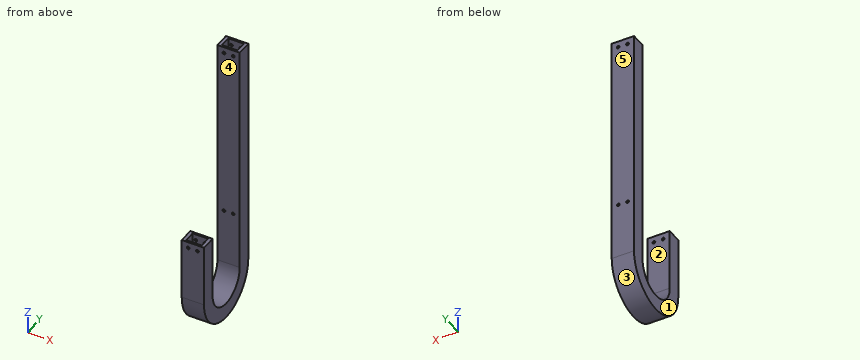
```python
from build123d import *

# Parameters (mm, degrees)
SKETCH_2_W          = 36
SKETCH_2_H          = 24
SKETCH_2_W_2        = 25
SKETCH_2_H_2        = 18
SKETCH_4_R          = 2.25
CUT_EXTRUDE_1_DEPTH = 304.110540892


with BuildPart() as part:
    # 扫描1: sweep along a path in 草图3
    with BuildLine(Plane(origin=(0, 0, 0), x_dir=(0, 0, -1), z_dir=(1, 0, 0))) as sweep_1_path:
        Line((0, 0), (100, 0))
        ThreePointArc((100, 0), (150, 50), (100, 100))
        Line((100, 100), (-276, 100))
    # 草图2 → 扫描1 (sweep)
    with BuildSketch(Plane.XY):
        Rectangle(SKETCH_2_W, SKETCH_2_H)
        Rectangle(SKETCH_2_W_2, SKETCH_2_H_2, mode=Mode.SUBTRACT)
    sweep(path=sweep_1_path.line)

    # 草图4 → 切除-拉伸1 (cut, through all)
    with BuildSketch(Plane.XZ.offset(12)):
        with Locations(Location((-7.5, -10, 0), (0, 0, 180))):
            Circle(SKETCH_4_R)
        with Locations(Location((7.5, -10, 0), (0, 0, 180))):
            Circle(SKETCH_4_R)
        with Locations(Location((-7.5, 266, 0), (0, 0, 270))):
            Circle(SKETCH_4_R)
        with Locations(Location((7.5, 266, 0), (0, 0, 270))):
            Circle(SKETCH_4_R)
    extrude(amount=-CUT_EXTRUDE_1_DEPTH, mode=Mode.SUBTRACT)


solid = part.part
```
Could you check a few things on this model? Use its own coordinates, in mm. Face numbers are marked on the shaded views. A direction names the side the tool comes from. Round coordinates to 2 decimals unless told otherwise and drop trailing zeros. Loops run counter-clockwise (first coordinate to the right, second up) from the corner with the lowest first, then second, coordinate; pieces in that order, holes last. Notation, with made-up numbers: M 20.25,23.5 L 45.25,23.5 A14 cw 45.25,36.5 Z; hole C -17,5 d5. An arc over 180 degrees is marked long. Answer as CSV lines item,"result".
1) Imagine slicing it at C-C on z = 244.5. List the corners of the cut face in (x, y) for me.
From the geometry:
outline,"M -18,88 L 18,88 L 18,112 L -18,112 Z; hole M -12.5,91 L 12.5,91 L 12.5,109 L -12.5,109 Z"
2) Which directions (+Z, -Z, +X, -X, +Y, -Y) give clear straight access to the entire face, cutting with the end or side of a thin tool? Please do the marked faces 1 and 2.
From the geometry:
face 1,"+Z, -Z, -X, +Y, -Y"
face 2,"+Z, +X, -X"
3) Imagine slicing it at D-D on y = -3. List the corners of the cut face in (x, z) for me, and give its area (3 significant figures).
From the geometry:
outline,"M -18,-132.17 L 18,-132.17 L 18,0 L 12.5,0 L 12.5,-125.92 L -12.5,-125.92 L -12.5,0 L -18,0 Z"
area,"1,610 mm^2"
4) Imagine slicing it at A-A on z = -45. List the corners of the cut face in (x, y) for me, and give its area (3 significant figures).
From the geometry:
outline,"M -18,-12 L 18,-12 L 18,12 L -18,12 Z; M -18,88 L 18,88 L 18,112 L -18,112 Z; hole M -12.5,-9 L 12.5,-9 L 12.5,9 L -12.5,9 Z; hole M -12.5,91 L 12.5,91 L 12.5,109 L -12.5,109 Z"
area,"828 mm^2"
5) Imagine slicing it at B-B on y = 50. List the corners of the cut face in (x, z) for me.
From the geometry:
outline,"M -18,-162 L 18,-162 L 18,-138 L -18,-138 Z; hole M -12.5,-159 L 12.5,-159 L 12.5,-141 L -12.5,-141 Z"
6) If I drill on probe 1 along X at (y, z) = (11.3, -10); probe 2 along Y at (x, z) = (-6, -72); probe 3 along X at (y, z) = (97, 257.5), over which ranges is the centre line in solid material (lowest first)?
From the geometry:
probe 1,"-18 to -9.75, -5.25 to 5.25, 9.75 to 18"
probe 2,"-12 to -9, 9 to 12, 88 to 91, 109 to 112"
probe 3,"-18 to -12.5, 12.5 to 18"
7) For pin 1 Ø1.5 at (x, y) = (9, 64) entering from +Z; pin 2 Ø8 at (x, y) = (11, 99) entering from -Z; pin 3 Ø7.5 at (x, z) = (-2.5, 128.5) entering from -Y; pin 4 Ø1 at (y, z) = (86, -80) entering from -X, each with a flat end and sliding along its axis, tell me the tip position at first contact or that it passes through.
From the geometry:
pin 1,"z = -135.02"
pin 2,"z = -142.65"
pin 3,"y = 88"
pin 4,"through"
8) We'd pull the mould along Y, two halves only. Please class the marked faces 3, 4 and 5: released by +Y, released by -Y, zero draft, split by the parting line, or undercut.
From the geometry:
face 3,"split by the parting line"
face 4,"undercut"
face 5,"released by +Y"
